Input: part model. Units: mm. Frame: model coordinates. A direction names the side the tool comes from. Coordinates: 2 decimals unless noted, no trailing zeros. Loops run counter-clockwise (first coordinate to the right, second up) from the corner with the lowest first, then second, coordinate; pieces in that order, holes last. Notation, with made-up numbers: M -28,67 L 17,67 A16 cw 17,98 Z; hole C 43,51.25 d3. An arc over 180 degrees is marked long. Use a Markdown table: item, result. Add a question column.
1. Section C-C on y = 23. Output: boundary loops of the cut face in (x, z), then the cut area to 3 significant figures.
2. Section A-A on z = -26.5. Output: boundary loops of the cut face in (x, y).
3. Line query: L1, parallel to X at y = 5.75, z = -34.72; L2, parallel to Y at x = 4.5, z = -38.5; L3, parallel to X at y = 9.75, z = -15. Output: solid intervals per line, ascending. Write a range as [from, to].
4. Draft query along X for faces 4 (the cylindrical face through (-6.56, 12.32, 4.58)), 5 (the cylindrical face through (-1.532, 20.07, -31.025)), 6 (the flat face through (17, 0, 1)). Return one class per face: +X half, -X half, draft (parallel to the pull), parting line (faces both ways), or undercut.
5. Section B-B on x = 52.5. Output: boundary loops of the cut face in (y, z).
6. Pin query (flat end, axial travel): pin 1 (10.5 mm diameter, centred on x = 0, z = -34.72, fed in from -Y); pin 2 (2 mm diameter, centred on x = 29.5, y = 5.5, fed in from -Z); pin 3 (8 mm diameter, centred on y = 7, z = -16, fed in from +X); pin 4 (6 mm diameter, centred on x = 34.5, y = 7.5, fed in from +Z). Return the tip coordinate at first contact, or that it passes through.
7. Section D-D on x = 0. Output: boundary loops of the cut face in (y, z).
8. Set-up query: faces 1 (the flat face through (8, 9.5, -20.3)), 2 (the flat face through (0, 12, -17.57)), 3 (the flat face through (24.624, 12.325, 18.057)). Return all of +Z, -Z, +X, -X, +Y, -Y with unobstructed straight access to the full face (end or side cutting, diameter ignored); none if empty.
```python
from build123d import *

# Parameters (mm, degrees)
L_BRACKET_BODY_DEPTH   = 25
PIVOT_HOLES_SKETCH_R   = 4
PIVOT_HOLES_3X_8_DEPTH = 25
CLEVIS_SLOT_SKETCH_W   = 25.15
CLEVIS_SLOT_SKETCH_H   = 5
CLEVIS_SLOT_5MM_DEPTH  = 12.5


with BuildPart() as part:
    # Bracket Profile Sketch → L Bracket Body (new body)
    with BuildSketch(Plane(origin=(0, 0, 0), x_dir=(1, 0, 0), z_dir=(0, 1, 0))):
        with BuildLine():
            Line((8, 34.72), (8, 5.491702761))
            Line((8, 5.491702761), (57.11524489, -13.424548452))
            ThreePointArc((57.11524489, -13.424548452), (61.705451548, -23.76524489), (51.36475511, -28.355451548))
            Line((51.36475511, -28.355451548), (-2.87524489, -7.465451548))
            ThreePointArc((-2.87524489, -7.465451548), (-6.595527239, -4.527584393), (-8, 0))
            Line((-8, 0), (-8, 34.72))
            ThreePointArc((-8, 34.72), (0, 42.72), (8, 34.72))
        make_face()
    extrude(amount=L_BRACKET_BODY_DEPTH)

    # Pivot Holes Sketch → Pivot Holes 3xØ8 (cut)
    with BuildSketch(Plane(origin=(0, 25, 0), x_dir=(1, 0, 0), z_dir=(0, 1, 0))):
        with Locations(Location((0, 34.72, 0), (0, 0, 270))):
            Circle(PIVOT_HOLES_SKETCH_R)
        with Locations(Location((54.24, -20.89, 0), (0, 0, 270))):
            Circle(PIVOT_HOLES_SKETCH_R)
        with Locations(Location((0, 0, 0), (0, 0, 270))):
            Circle(PIVOT_HOLES_SKETCH_R)
    extrude(amount=-PIVOT_HOLES_3X_8_DEPTH, mode=Mode.SUBTRACT)

    # Clevis Slot Sketch → Clevis Slot 5mm (cut, symmetric)
    with BuildSketch(Plane(origin=(0, 0, 0), x_dir=(0, 0, -1), z_dir=(1, 0, 0))):
        with Locations((30.145, 12.5)):
            Rectangle(CLEVIS_SLOT_SKETCH_W, CLEVIS_SLOT_SKETCH_H)
    extrude(amount=CLEVIS_SLOT_5MM_DEPTH, both=True, mode=Mode.SUBTRACT)


solid = part.part
```
Answers below:
| question | item | result |
|---|---|---|
| 1 | outline | M -8,-34.72 A8 ccw 8,-34.72 L 8,-5.49 L 57.12,13.42 A8 ccw 51.36,28.36 L -2.88,7.47 A8 ccw -8,0 Z; hole C 0,-34.72 d8; hole C 0,0 d8; hole C 54.24,20.89 d8 |
| 1 | area | 1,530 mm² |
| 2 | outline | M -8,0 L 8,0 L 8,10 L -8,10 Z; M -8,15 L 8,15 L 8,25 L -8,25 Z |
| 3 | L1 | x = [-8, -4], [4, 8] |
| 3 | L2 | y = [0, 10], [15, 25] |
| 3 | L3 | x = [-8, 8] |
| 4 | face 4 | -X half |
| 4 | face 5 | undercut |
| 4 | face 6 | draft |
| 5 | outline | M 0,11.65 L 25,11.65 L 25,17.29 L 0,17.29 Z; M 0,24.49 L 25,24.49 L 25,28.7 L 0,28.7 Z |
| 6 | pin 1 | stops at y = 0 |
| 6 | pin 2 | stops at z = 2.4 |
| 6 | pin 3 | stops at x = 8 |
| 6 | pin 4 | stops at z = 23.02 |
| 7 | outline | M 0,-42.72 L 10,-42.72 L 10,-38.72 L 0,-38.72 Z; M 0,-30.72 L 10,-30.72 L 10,-17.57 L 15,-17.57 L 15,-30.72 L 25,-30.72 L 25,-4 L 0,-4 Z; M 0,4 L 25,4 L 25,8.57 L 0,8.57 Z; M 15,-42.72 L 25,-42.72 L 25,-38.72 L 15,-38.72 Z |
| 8 | face 1 | -Z, +X, +Y, -Y |
| 8 | face 2 | -Z, +X, -X |
| 8 | face 3 | +Z, -X, +Y, -Y |
